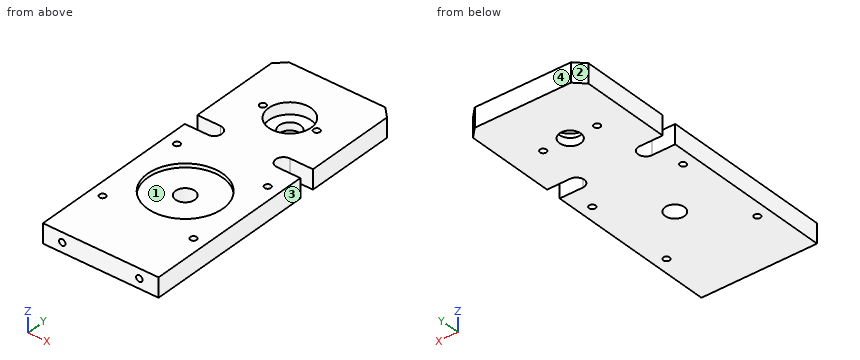
```python
from build123d import *

# Parameters (mm, degrees)
SKETCH1_W             = 60
SKETCH1_H             = 150
BOSS_EXTRUDE1_DEPTH   = 10
CHAMFER1_SIZE         = 5
CUT_EXTRUDE5_START    = -10
SKETCH5_R             = 19.5
CUT_EXTRUDE5_DEPTH    = 2
SKETCH6_R             = 5
CUT_EXTRUDE6_DEPTH    = 82.172655494
M4_TAPPED_HOLE1_D     = 3.3
SKETCH9_R             = 11
CUT_EXTRUDE7_DEPTH    = 6
SKETCH10_R            = 5.5
CUT_EXTRUDE8_DEPTH    = 82
CUT_EXTRUDE9_DEPTH    = 82.39410298
M4_TAPPED_HOLE2_D     = 3.3
M4_TAPPED_HOLE3_D     = 3.3
M4_TAPPED_HOLE3_DEPTH = 11.5
M4_TAPPED_HOLE3_TIP   = 0.991420021


with BuildPart() as part:
    # Sketch1 → Boss-Extrude1 (new body)
    with BuildSketch(Plane.XY):
        Rectangle(SKETCH1_W, SKETCH1_H)
    extrude(amount=BOSS_EXTRUDE1_DEPTH)

    # Chamfer1
    chamfer1_edges = [part.edges().sort_by_distance(p)[0] for p in [
        (-30, 75, 5),
        (30, 75, 5),
    ]]
    chamfer(chamfer1_edges, length=CHAMFER1_SIZE)

    # Sketch5 → Cut-Extrude5 (cut)
    with BuildSketch(Plane(origin=(0, 0, 0), x_dir=(-1, 0, 0), z_dir=(0, 0, -1)).offset(CUT_EXTRUDE5_START)):
        with Locations((0, -21.425)):
            Circle(SKETCH5_R)
    extrude(amount=CUT_EXTRUDE5_DEPTH, mode=Mode.SUBTRACT)

    # Sketch6 → Cut-Extrude6 (cut, through all)
    with BuildSketch(Plane.XY.offset(8)):
        with Locations((0, -21.425)):
            Circle(SKETCH6_R)
    extrude(amount=-CUT_EXTRUDE6_DEPTH, mode=Mode.SUBTRACT)

    # M4 Tapped Hole1 (through all)
    with Locations(Plane.XY.offset(10)):
        with Locations((-23.57, 2.145), (-23.57, -44.995), (23.57, 2.145), (23.57, -44.995)):
            Hole(M4_TAPPED_HOLE1_D / 2)

    # Sketch9 → Cut-Extrude7 (cut)
    with BuildSketch(Plane.XY.offset(10)):
        with Locations((0, 45)):
            Circle(SKETCH9_R)
    extrude(amount=-CUT_EXTRUDE7_DEPTH, mode=Mode.SUBTRACT)

    # Sketch10 → Cut-Extrude8 (cut, through all)
    with BuildSketch(Plane.XY.offset(4)):
        with Locations((0, 45)):
            Circle(SKETCH10_R)
    extrude(amount=-CUT_EXTRUDE8_DEPTH, mode=Mode.SUBTRACT)

    # Sketch11 → Cut-Extrude9 (cut, through all)
    with BuildSketch(Plane(origin=(0, 0, 0), x_dir=(-1, 0, 0), z_dir=(0, 0, -1))):
        with BuildLine():
            Line((18, 23), (40.992730917, 23))
            ThreePointArc((40.992730917, 23), (44.992730917, 19), (40.992730917, 15))
            Line((40.992730917, 15), (18, 15))
            ThreePointArc((18, 15), (14, 19), (18, 23))
        make_face()
    cut_extrude9 = extrude(amount=-CUT_EXTRUDE9_DEPTH, mode=Mode.SUBTRACT)

    # Mirror1: Cut-Extrude9 across plane
    add(cut_extrude9.mirror(Plane(origin=(0, 0, 0), x_dir=(0, 0, 1), z_dir=(1, 0, 0))), mode=Mode.SUBTRACT)

    # M4 Tapped Hole2 (through all)
    with Locations(Plane.XY.offset(10)):
        with Locations((-14, 45), (14, 45)):
            Hole(M4_TAPPED_HOLE2_D / 2)

    # M4 Tapped Hole3
    with Locations(Plane(origin=(0, -75, 0), x_dir=(-1, 0, 0), z_dir=(0, -1, 0))):
        with Locations((20, -5), (-20, -5)):
            Hole(M4_TAPPED_HOLE3_D / 2, depth=M4_TAPPED_HOLE3_DEPTH)
            with Locations((0, 0, -(M4_TAPPED_HOLE3_DEPTH + M4_TAPPED_HOLE3_TIP / 2))):  # 118° drill point
                Cone(0, M4_TAPPED_HOLE3_D / 2, M4_TAPPED_HOLE3_TIP, mode=Mode.SUBTRACT)


solid = part.part
```
Read the model definition and answer for the solid it produces. Units are mm, in the model's axes. Face numbers are marked on the shaded views. Coordinates: 2 decimals unless noted, no trailing zeros. Order: outer loops, then holes, each group sorted by start corner. A loop starts at its lowest first (then second) coordinate and runs counter-clockwise, first axis right, second up. Notation, with made-up numbers: (46, -35) - (70, -35) arc R25 cw to (70, -20) - close; hole circle Ø5 at (-33.75, 61.5). An arc over 180 degrees is marked (long way). Answer as a JSON object with one key per item and string values. Group by question number.
Item 1: Consider probe 1 along Y at (x, z) = (-23.57, 6.75) (3 decimals); probe 2 along Y at (x, z) = (0, 8.65) (3 decimals); probe 3 along Y at (x, z) = (-21, 1.5). Determine where each line is inside the solid, lowest interval first. Write a range as from..to.
Item 2: Section C-C (x = 0) is taken. Give the vertices of the cut face in (y, z) (3 decimals), plus the area to 3 significant figures.
Item 3: Flat-ended cylindrical pins translate along their axes: P1, Ø20, axis at x = 0, y = 45, coming from the +Z side; P2, Ø11.5, axis at x = -7, y = -14.5, coming from the +Z side; P3, Ø2.5, axis at x = -23.57, y = 2.145, coming from the -Z side. Find the tip coordinate at first contact, or state that the pin passes through.
Item 4: Section B-B (x = -23.57) is taken. Give the vertices of the cut face in (y, z) (3 decimals).
Item 5: Section A-A (y = 45) is taken. Give the vertices of the cut face in (x, z).
Item 6: The mould has two halves that part along X. Classify the marked faces 1, 2, 3 and 4: +X half, -X half, draft (parallel to the pull), parting line (faces both ways), or undercut.
Results are:
{
 "1": {"probe 1": "y = -75..-46.645, -43.345..0.495, 3.795..15, 23..75", "probe 2": "y = -75..-40.925, -1.925..34, 56..75", "probe 3": "y = -75..15, 23..75"},
 "2": {"outline": "(-75, 0) - (-26.425, 0) - (-26.425, 8) - (-40.925, 8) - (-40.925, 10) - (-75, 10) - close; (-16.425, 0) - (39.5, 0) - (39.5, 4) - (34, 4) - (34, 10) - (-1.925, 10) - (-1.925, 8) - (-16.425, 8) - close; (50.5, 0) - (75, 0) - (75, 10) - (56, 10) - (56, 4) - (50.5, 4) - close", "area": "1,170 mm^2"},
 "3": {"P1": "stops at z = 4", "P2": "stops at z = 8", "P3": "passes through"},
 "4": {"outline": "(-75, 0) - (-46.645, 0) - (-46.645, 10) - (-75, 10) - close; (-43.345, 0) - (0.495, 0) - (0.495, 10) - (-43.345, 10) - close; (3.795, 0) - (15, 0) - (15, 10) - (3.795, 10) - close; (23, 0) - (75, 0) - (75, 10) - (23, 10) - close"},
 "5": {"outline": "(-30, 0) - (-15.65, 0) - (-15.65, 10) - (-30, 10) - close; (-12.35, 0) - (-5.5, 0) - (-5.5, 4) - (-11, 4) - (-11, 10) - (-12.35, 10) - close; (5.5, 0) - (12.35, 0) - (12.35, 10) - (11, 10) - (11, 4) - (5.5, 4) - close; (15.65, 0) - (30, 0) - (30, 10) - (15.65, 10) - close"},
 "6": {"face 1": "undercut", "face 2": "-X half", "face 3": "+X half", "face 4": "draft"}
}
